Source: three-view drawing plus pictorial views. Frame: mm from the lowest corner of the part. Give positions to 0.01 mm unless a question says otherwise; leave off trailing zeros. Write each loop counter-clockwise with the first axis right and the second up, starting at its lowest first coordinate (ties: lowest second). Pieces come first, ordered by that corner, then holes. Notation, with made-up numbers: M 72.25,73 L 89.25,73 A20 ccw 89.25,80 Z; hole C 41.5,-5 d10. An arc over 180 degrees is marked long. Return JSON: item names as keys, results as strings.
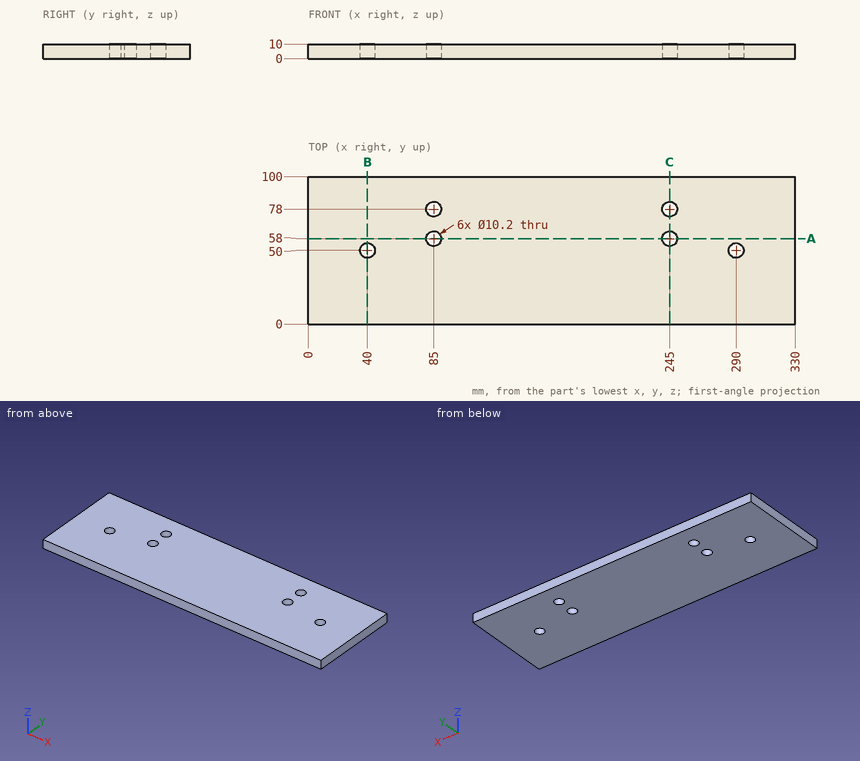
1) Cut plane B-B, the plane x = 40. Return the cut outline in (y, z), then the cut area to 3 significant figures.
Numbers:
{"outline": "M 0,0 L 44.9,0 L 44.9,10 L 0,10 Z; M 55.1,0 L 100,0 L 100,10 L 55.1,10 Z", "area": "898 mm²"}
2) Cut plane C-C, the plane x = 245. Return the cut outline in (y, z), then the cut area to 3 significant figures.
Numbers:
{"outline": "M 0,0 L 52.9,0 L 52.9,10 L 0,10 Z; M 63.1,0 L 72.9,0 L 72.9,10 L 63.1,10 Z; M 83.1,0 L 100,0 L 100,10 L 83.1,10 Z", "area": "796 mm²"}
3) Cut plane A-A, the plane y = 58. Return the cut outline in (x, z).
Numbers:
{"outline": "M 0,0 L 79.9,0 L 79.9,10 L 0,10 Z; M 90.1,0 L 239.9,0 L 239.9,10 L 90.1,10 Z; M 250.1,0 L 330,0 L 330,10 L 250.1,10 Z"}
4) Contact query for a flat-ended pin moving along its axis: pin 1 Ø9 at (x, y) = (85, 58) entering from -Z. Output: stop coordinate, or through.
Numbers:
{"pin 1": "passes through"}
5) Line query: line 1 (Y direction, x = 245, z = 3.5); line 2 (Y direction, x = 40, z = 7.25); line 3 (X direction, y = 51, z = 2.5). Output: solid intervals per line, ascending. Write a range as [from, to].
Numbers:
{"line 1": "y = [0, 52.9], [63.1, 72.9], [83.1, 100]", "line 2": "y = [0, 44.9], [55.1, 100]", "line 3": "x = [0, 35], [45, 285], [295, 330]"}
